Part model, mm, in its own coordinate system. Face numbers are marked on the shaded views. A direction names the side the tool comes from. Give positions to 0.01 mm unless a question says otherwise; leave off trailing zeros. Write each loop counter-clockwise with the first axis right and the second up, starting at its lowest first coordinate (ties: lowest second). Pieces come first, ordered by that corner, then holes.
from build123d import *

# Parameters (mm, degrees)
SKETCH3_R          = 57.15
CUT_EXTRUDE1_DEPTH = 50


with BuildPart() as part:
    # Sweep1: sweep along a path in Sketch2
    with BuildLine(Plane(origin=(0, 0, 0), x_dir=(0, 0, -1), z_dir=(1, 0, 0))) as sweep1_path:
        ThreePointArc((0, 20.7), (-715, -158.48445696), (-1260.994295686, -653.683708467))
    # Sketch1 → Sweep1 (sweep)
    with BuildSketch(Plane.XY):
        with BuildLine():
            Line((-158.75, 20.7), (-53.975, 20.7))
            ThreePointArc((-53.975, 20.7), (-48.941078797, 19.961460685), (-44.331437049, 17.808089852))
            Line((-44.331437049, 17.808089852), (-5.241365883, -7.953220019))
            ThreePointArc((-5.241365883, -7.953220019), (0, -9.525), (5.241365883, -7.953220019))
            Line((5.241365883, -7.953220019), (44.331437049, 17.808089852))
            ThreePointArc((44.331437049, 17.808089852), (48.941078797, 19.961460685), (53.975, 20.7))
            Line((53.975, 20.7), (158.75, 20.7))
            Line((158.75, 20.7), (158.75, 12.7))
            Line((158.75, 12.7), (53.975, 12.7))
            ThreePointArc((53.975, 12.7), (51.23901715, 12.298597034), (48.733634117, 11.128220019))
            Line((48.733634117, 11.128220019), (9.643562951, -14.633089852))
            ThreePointArc((9.643562951, -14.633089852), (0, -17.525), (-9.643562951, -14.633089852))
            Line((-9.643562951, -14.633089852), (-48.733634117, 11.128220019))
            ThreePointArc((-48.733634117, 11.128220019), (-51.23901715, 12.298597034), (-53.975, 12.7))
            Line((-53.975, 12.7), (-158.75, 12.7))
            Line((-158.75, 12.7), (-158.75, 20.7))
        make_face()
    sweep(path=sweep1_path.line)

    # Sketch3 → Cut-Extrude1 (cut, symmetric)
    with BuildSketch(Plane(origin=(0, 0, 0), x_dir=(1, 0, 0), z_dir=(0, 1, 0))):
        Circle(SKETCH3_R)
    extrude(amount=CUT_EXTRUDE1_DEPTH, both=True, mode=Mode.SUBTRACT)


solid = part.part
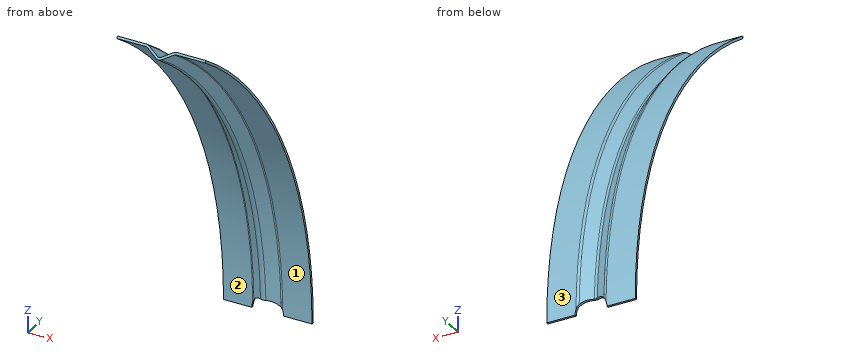
1) 3-axis set-ups, long thin cutter, end or side, ignore diameter. For the marked faces 1, 2 and 3: which of +Z, -Z, +X, -X, +Y, -Y reach the whole face in a straight line?
Check result:
face 1: -Z, +X, -Y
face 2: -Z, -X, -Y
face 3: +Z, +X, -X, +Y
2) Saw through at A-A (x = 21.5). Write the cut outline in (y, z) (3 decimals), and give its area (3 significant figures).
Check result:
outline: (-668.962, 1238.106) arc R1488.606 cw to (-7.761, 52.952) - (1.826, 52.952) arc R1498.187 ccw to (-663.643, 1246.075) - close
area: 13,500 mm2
3) Flat gauge pins, fed straight in: P1, Ø1, axis at x = -54.5, y = -320, coming from the -Z side; P2, Ø10, axis at x = 120, y = -368.5, coming from the -Z side; P3, Ø1, axis at x = 79.5, y = -138.5, coming from the -Z side. Where does each tip first touch, or does it go through?
Check result:
P1: stops at z = 944.27
P2: stops at z = 996.59
P3: stops at z = 657.14
4) Drill centre lines: L1, parallel to Y at x = -58, z = 522.5; L2, parallel to Z at x = -117, y = -123.5; L3, parallel to Y at x = 126.5, z = 1017. Where is each one in solid material? Low to high.
Check result:
L1: y = -80.7 to -72.18
L2: z = 626.31 to 645.33
L3: y = -381.8 to -370.99
